The listing builds one solid part. Answer for the finished solid, in the listing's coordinates (mm). A direction names the side the tool comes from. Give positions to 0.01 mm unless a question says otherwise; leave off trailing zeros. Order: outer loops, then holes, each group sorted by start corner. A loop starts at its lowest first (then second) coordinate and runs counter-clockwise, first axis right, second up.
```python
from build123d import *

# Parameters (mm, degrees)
SKETCH1_R               = 40
BOSS_EXTRUDE1_DEPTH     = 30
SKETCH2_R               = 18
BOSS_EXTRUDE2_DEPTH     = 60
SKETCH3_W               = 77.976815456
SKETCH3_H               = 25.992271819
SKETCH3_W_2             = 92.098600933
SKETCH3_H_2             = 25.173617588
CUT_EXTRUDE1_DEPTH      = 18
SKETCH7_R               = 42.5
BOSS_EXTRUDE3_DEPTH     = 38
SKETCH14_R              = 3
CUT_EXTRUDE3_DEPTH      = 63
CUT_EXTRUDE4_START      = -30
SKETCH15_R              = 67.080871601
SKETCH15_R_2            = 40
CUT_EXTRUDE4_DEPTH      = 3
SKETCH17_R              = 45
SKETCH17_R_2            = 16.642095107
BOSS_EXTRUDE4_DEPTH     = 10
CHAMFER1_SIZE           = 1
CUT_EXTRUDE5_DEPTH      = 111.227038425
CUT_EXTRUDE5_DEPTH_BACK = 111.227038425
SKETCH20_R              = 45
BOSS_EXTRUDE5_DEPTH     = 2
CHAMFER2_SIZE           = 1
CHAMFER3_SIZE           = 1
SKETCH21_R              = 3
CUT_EXTRUDE7_DEPTH      = 2
SKETCH22_R              = 18
CUT_EXTRUDE8_DEPTH      = 94.134311615
M52X5_0_TAPPED_HOLE1_D  = 47
BOSS_EXTRUDE6_START     = -33
SKETCH25_R              = 42.5
SKETCH25_R_2            = 34.471384151
BOSS_EXTRUDE6_DEPTH     = 33
SKETCH26_OUTSIDE_W      = 120.862
SKETCH26_OUTSIDE_H      = 120.862
SKETCH26_OUTSIDE_R      = 40
CUT_EXTRUDE9_DEPTH      = 3
CHAMFER4_SIZE           = 0.5
M6_TAPPED_HOLE1_D       = 5
M6_TAPPED_HOLE1_DEPTH   = 17
M6_TAPPED_HOLE1_TIP     = 1.502151548


with BuildPart() as part:
    # Sketch1 → Boss-Extrude1 (new body)
    with BuildSketch(Plane(origin=(0, 0, 0), x_dir=(1, 0, 0), z_dir=(0, 1, 0))):
        with Locations(Location((0, 0, 0), (0, 0, 270))):
            Circle(SKETCH1_R)
    extrude(amount=BOSS_EXTRUDE1_DEPTH)

    # Sketch2 → Boss-Extrude2 (add)
    with BuildSketch(Plane(origin=(0, 30, 0), x_dir=(1, 0, 0), z_dir=(0, 1, 0))):
        with Locations(Location((0, 0, 0), (0, 0, 270))):
            Circle(SKETCH2_R)
    extrude(amount=BOSS_EXTRUDE2_DEPTH)

    # Sketch3 → Cut-Extrude1 (cut)
    with BuildSketch(Plane(origin=(0, 30, 0), x_dir=(1, 0, 0), z_dir=(0, 1, 0))):
        with Locations((-2.353630913, 48.996135909)):
            Rectangle(SKETCH3_W, SKETCH3_H)
        with Locations((4.707261826, -48.586808794)):
            Rectangle(SKETCH3_W_2, SKETCH3_H_2)
    extrude(amount=-CUT_EXTRUDE1_DEPTH, mode=Mode.SUBTRACT)

    # Sketch7 → Boss-Extrude3 (add)
    with BuildSketch(Plane.XZ):
        with Locations(Location((0, 0, 0), (0, 0, 270))):
            Circle(SKETCH7_R)
    extrude(amount=BOSS_EXTRUDE3_DEPTH)

    # Sketch14 → Cut-Extrude3 (cut)
    with BuildSketch(Plane.XZ.offset(38)):
        with Locations(Location((0, 0, 0), (0, 0, 270))):
            Circle(SKETCH14_R)
    extrude(amount=-CUT_EXTRUDE3_DEPTH, mode=Mode.SUBTRACT)

    # Sketch15 → Cut-Extrude4 (cut)
    with BuildSketch(Plane.XZ.offset(38).offset(CUT_EXTRUDE4_START)):
        Circle(SKETCH15_R)
        with Locations(Location((0, 0, 0), (0, 0, 270))):
            Circle(SKETCH15_R_2, mode=Mode.SUBTRACT)
    extrude(amount=-CUT_EXTRUDE4_DEPTH, mode=Mode.SUBTRACT)

    # Sketch17 → Boss-Extrude4 (add)
    with BuildSketch(Plane.XZ.offset(5)):
        with Locations(Location((0, 0, 0), (0, 0, 270))):
            Circle(SKETCH17_R)
        Circle(SKETCH17_R_2, mode=Mode.SUBTRACT)
    extrude(amount=-BOSS_EXTRUDE4_DEPTH)

    # Chamfer1
    chamfer1_edges = [part.edges().sort_by_distance(p)[0] for p in [
        (40, 30, 0),
        (0, -38, 42.5),
        (0, -5, 45),
        (0, 90, -18),
        (-40, 30, 0),
    ]]
    chamfer(chamfer1_edges, length=CHAMFER1_SIZE)

    # Sketch18 → Cut-Extrude5 (cut, two sides: drawn at the far end of the back side and taken through both)
    with BuildSketch(Plane(origin=(0, 0, 0), x_dir=(0, 0, -1), z_dir=(1, 0, 0)).offset(-CUT_EXTRUDE5_DEPTH_BACK)):
        Polygon((-40, 12), (-40, 8), (-36, 12), align=None)
        Polygon((36, 12), (41.96059215, 12), (41.96059215, 6.03940785), align=None)
    extrude(amount=CUT_EXTRUDE5_DEPTH + CUT_EXTRUDE5_DEPTH_BACK, mode=Mode.SUBTRACT)

    # Sketch20 → Boss-Extrude5 (add)
    with BuildSketch(Plane(origin=(0, 5, 0), x_dir=(1, 0, 0), z_dir=(0, 1, 0))):
        with Locations(Location((0, 0, 0), (0, 0, 90))):
            Circle(SKETCH20_R)
    extrude(amount=BOSS_EXTRUDE5_DEPTH)

    # Chamfer2
    chamfer2_edges = [part.edges().sort_by_distance(p)[0] for p in [
        (0, 7, 45),
    ]]
    chamfer(chamfer2_edges, length=CHAMFER2_SIZE)

    # Chamfer3
    chamfer3_edges = [part.edges().sort_by_distance(p)[0] for p in [
        (0, -8, 42.5),
    ]]
    chamfer(chamfer3_edges, length=CHAMFER3_SIZE)

    # Sketch21 → Cut-Extrude7 (cut)
    with BuildSketch(Plane.XZ.offset(-5)):
        with Locations(Location((0, 0, 0), (0, 0, 270))):
            Circle(SKETCH21_R)
    extrude(amount=-CUT_EXTRUDE7_DEPTH, mode=Mode.SUBTRACT)

    # Sketch22 → Cut-Extrude8 (cut, through all)
    with BuildSketch(Plane(origin=(0, 30, 0), x_dir=(1, 0, 0), z_dir=(0, 1, 0))):
        Circle(SKETCH22_R)
    extrude(amount=CUT_EXTRUDE8_DEPTH, mode=Mode.SUBTRACT)

    # M52x5.0 Tapped Hole1 (through all)
    with Locations(Plane(origin=(0, 30, 0), x_dir=(1, 0, 0), z_dir=(0, 1, 0))):
        with Locations((0, 0)):
            Hole(M52X5_0_TAPPED_HOLE1_D / 2)

    # Sketch25 → Boss-Extrude6 (add)
    with BuildSketch(Plane.XZ.offset(38).offset(BOSS_EXTRUDE6_START)):
        with Locations(Location((0, 0, 0), (0, 0, 270))):
            Circle(SKETCH25_R)
        Circle(SKETCH25_R_2, mode=Mode.SUBTRACT)
    extrude(amount=BOSS_EXTRUDE6_DEPTH)

    # Sketch26 outside → Cut-Extrude9 (cut)
    with BuildSketch(Plane.XZ.offset(5)):
        Rectangle(SKETCH26_OUTSIDE_W, SKETCH26_OUTSIDE_H)
        with Locations(Location((0, 0, 0), (0, 0, 244.158067237))):
            Circle(SKETCH26_OUTSIDE_R, mode=Mode.SUBTRACT)
    extrude(amount=CUT_EXTRUDE9_DEPTH, mode=Mode.SUBTRACT)

    # Chamfer4
    chamfer4_edges = [part.edges().sort_by_distance(p)[0] for p in [
        (0, -38, 42.5),
        (0, -8, 42.5),
    ]]
    chamfer(chamfer4_edges, length=CHAMFER4_SIZE)

    # M6 Tapped Hole1
    with Locations(Plane.XY.offset(36)):
        with Locations((0, 21)):
            Hole(M6_TAPPED_HOLE1_D / 2, depth=M6_TAPPED_HOLE1_DEPTH)
            with Locations((0, 0, -(M6_TAPPED_HOLE1_DEPTH + M6_TAPPED_HOLE1_TIP / 2))):  # 118° drill point
                Cone(0, M6_TAPPED_HOLE1_D / 2, M6_TAPPED_HOLE1_TIP, mode=Mode.SUBTRACT)


solid = part.part
```
1) Straight lines are drawn through the part: probe 1 along Z at (x, y) = (0, -23); probe 2 along Y at (x, z) = (-34, 23); probe 3 along Y at (x, z) = (0, 32). For each, find the intervals that lie inside material, in ascending order.
Geometry says:
probe 1: z = -42.5 to -23.5, 23.5 to 42.5
probe 2: y = -38 to -8, -5 to 7
probe 3: y = -38 to 18.5, 23.5 to 30
2) Given P1, Ø5, axis at x = -25, y = -11.5, coming from the -Z side; P2, Ø9, axis at x = -7, y = 21.5, coming from the +Z side; P3, Ø8, axis at y = 6, z = -16.5, coming from the -X side, each flat-ended and moving along its own axis, determine where each tip first touches the part or whether it passes through.
Geometry says:
P1: stops at z = -36.06
P2: stops at z = 36
P3: stops at x = -43.23
3) For a pull along Y with two mould halves and no side action, classify faces 1 (the cylindrical face through (0.33, 23.48, 29.59)), 2 (the conical face through (39.154, 29.84, 0.645)), 3 (the flat face through (0, 21, -36)) as +Y half, -Y half, draft (parallel to the pull), parting line (faces both ways), or undercut.
Geometry says:
face 1: undercut
face 2: +Y half
face 3: draft
4) Find section C-C (x = 0). Count the separate pieces of the cut face and the enclosed holes in it, then the cut area to 3 significant figures.
Geometry says:
separate pieces: 3
enclosed holes: 0
area: 2,290 mm2
5) Find section B-B (y = 21). Write down the section's boundary in (x, z), then the cut area to 3 significant figures.
Geometry says:
outline: (-17.44, -36) - (17.44, -36) arc R40 ccw to (17.44, 36) - (2.5, 36) - (2.5, 23.37) arc R23.5 cw (long way) to (-2.5, 23.37) - (-2.5, 36) - (-17.44, 36) arc R40 ccw to start
area: 3,040 mm2
6) A tool of negligible diameter and unlimited length cuts with its end or side. For faces 4 (the cylindrical face through (-24, 18, -32)), 5 (the flat face through (37.1, -8, -15.4)), 6 (the flat face through (-4, 21, 36)), from which of +Z, -Z, +X, -X, +Y, -Y can it reach the whole face along a straight path? Write none if from no direction.
Geometry says:
face 4: +Y
face 5: none
face 6: +Z, +X, -X, +Y
